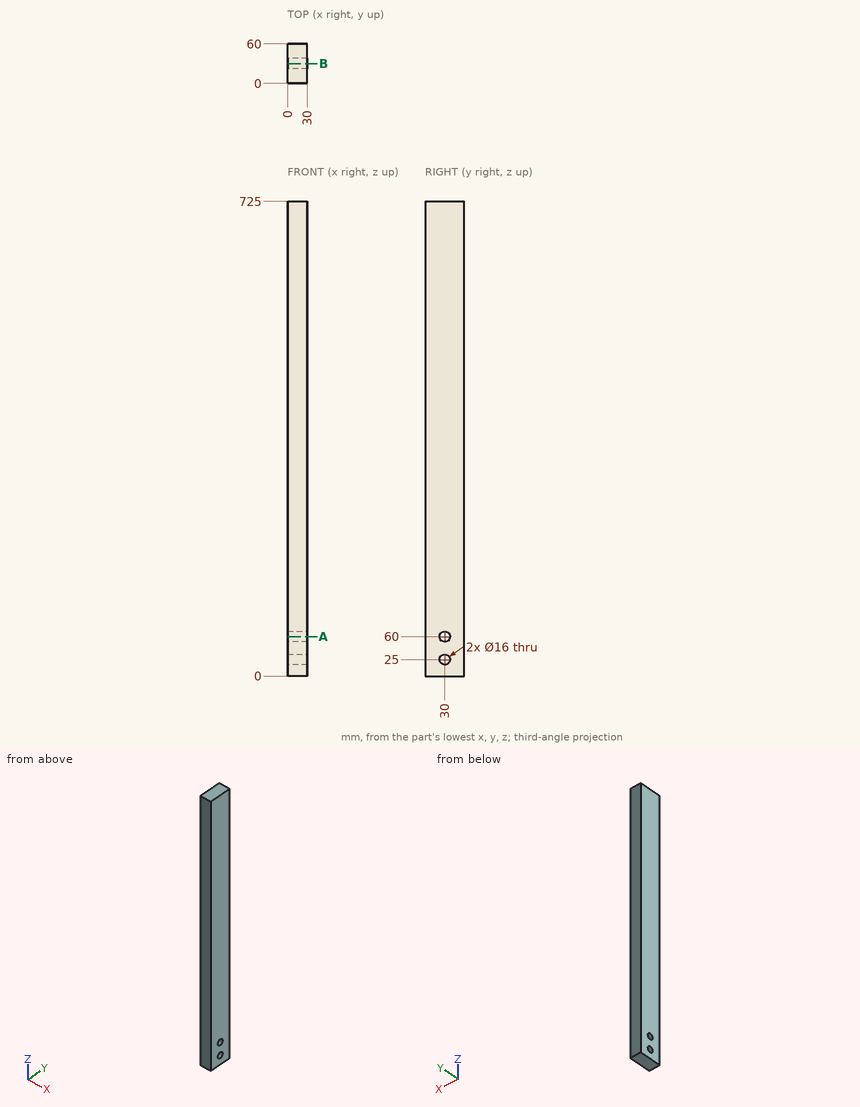
Job drawing, mm, ordinate dimensions from the low corner. One solid piece. Coordinates: 2 decimals unless noted, no trailing zeros. Loops run counter-clockwise (first coordinate to the right, second up) from the corner with the lowest first, then second, coordinate; pieces in that order, holes last. Notation, with made-up numbers: (22, 56) -> (59, 56) arc R11 ccw to (59, 64) -> close; hole circle Ø8 at (59, 81.5). An arc over 180 degrees is marked (long way). One line per item, written item: value.
1. Flat gauge pins, fed straight in: P1, Ø6, axis at x = 21, z = 619.5, coming from the -Y side; P2, Ø14.5, axis at y = 30, z = 60, coming from the +X side (3 decimals). Where does each tip first touch, or does it go through?
Answers:
P1: stops at y = 0
P2: passes through
2. Slice it at B-B on y = 30. Write the cut outline in (x, z), and give its area (3 significant figures).
Answers:
outline: (0, 0) -> (30, 0) -> (30, 17) -> (0, 17) -> close; (0, 33) -> (30, 33) -> (30, 52) -> (0, 52) -> close; (0, 68) -> (30, 68) -> (30, 725) -> (0, 725) -> close
area: 20,800 mm^2
3. Drill centre lines: line 1 (Y direction, x = 22.5, z = 25); line 2 (Z direction, x = 3, y = 34); line 3 (Y direction, x = 19.25, z = 30) (3 decimals). Where is each one in solid material? Low to high. Write a range as [from, to].
Answers:
line 1: y = [0, 22], [38, 60]
line 2: z = [0, 18.07], [31.93, 53.07], [66.93, 725]
line 3: y = [0, 23.755], [36.245, 60]
4. Slice it at A-A on z = 60. Write the cut outline in (x, y), and give its area (3 significant figures).
Answers:
outline: (0, 0) -> (30, 0) -> (30, 22) -> (0, 22) -> close; (0, 38) -> (30, 38) -> (30, 60) -> (0, 60) -> close
area: 1,320 mm^2
